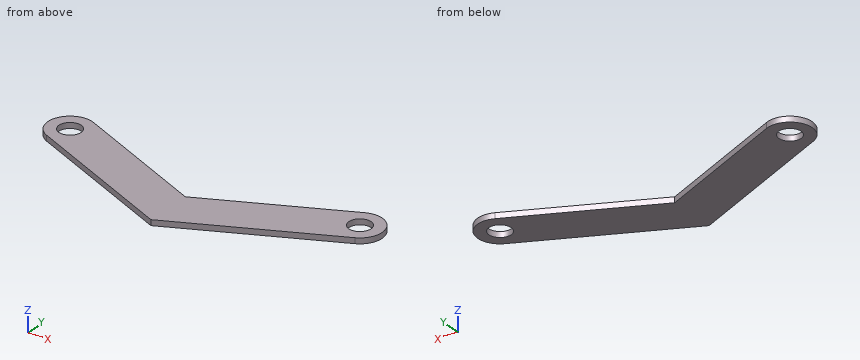
from build123d import *

# Parameters (mm, degrees)
SKETCH1_R           = 5
BOSS_EXTRUDE1_DEPTH = 2.5


with BuildPart() as part:
    # Sketch1 → Boss-Extrude1 (new body)
    with BuildSketch(Plane.XY):
        with BuildLine():
            Line((0, 21.995608), (61.387985551, 50.094742382))
            ThreePointArc((61.387985551, 50.094742382), (74.642724329, 45.164032502), (69.712014449, 31.909293724))
            Line((69.712014449, 31.909293724), (0, 0))
            Line((0, 0), (-69.712014449, 31.909293724))
            ThreePointArc((-69.712014449, 31.909293724), (-74.642724329, 45.164032502), (-61.387985551, 50.094742382))
            Line((-61.387985551, 50.094742382), (0, 21.995608))
        make_face()
        with Locations((-65.55, 41.002018053)):
            Circle(SKETCH1_R, mode=Mode.SUBTRACT)
        with Locations((65.55, 41.002018053)):
            Circle(SKETCH1_R, mode=Mode.SUBTRACT)
    extrude(amount=BOSS_EXTRUDE1_DEPTH)


solid = part.part
Geometry check sheet. Reference: the model listing, model coordinates, mm. Give positions to 0.01 mm unless a question says otherwise; leave off trailing zeros. Write each loop counter-clockwise with the first axis right and the second up, starting at its lowest first coordinate (ties: lowest second). Pieces come first, ordered by that corner, then holes.
1) Cross-section at B-B (z = 0.55). Record the boundary of the cut face in (x, y), plus the area to 3 significant figures.
Values follow:
outline: (-69.71, 31.91) - (0, 0) - (69.71, 31.91) arc R10 ccw to (61.39, 50.09) - (0, 22) - (-61.39, 50.09) arc R10 ccw to start; hole circle Ø10 at (-65.55, 41); hole circle Ø10 at (65.55, 41)
area: 3,040 mm2
2) Cross-section at D-D (x = -65.55). Record the boundary of the cut face in (y, z).
Values follow:
outline: (30, 0) - (36, 0) - (36, 2.5) - (30, 2.5) - close; (46, 0) - (51, 0) - (51, 2.5) - (46, 2.5) - close
3) Thickness scan on line 1 (X direction, y = 42, z = 0.85); line 2 (X direction, y = 47, z = 1.95); line 3 (Y direction, x = -65.55, z = 1.5). Record the ranges inside material, lowest first.
Values follow:
line 1: x = -75.5 to -70.45, -60.65 to -43.7, 43.7 to 60.65, 70.45 to 75.5
line 2: x = -73.55 to -54.63, 54.63 to 73.55
line 3: y = 30 to 36, 46 to 51
4) Cross-section at C-C (y = 44.5). Record the boundary of the cut face in (x, z).
Values follow:
outline: (-74.92, 0) - (-69.12, 0) - (-69.12, 2.5) - (-74.92, 2.5) - close; (-61.98, 0) - (-49.17, 0) - (-49.17, 2.5) - (-61.98, 2.5) - close; (49.17, 0) - (61.98, 0) - (61.98, 2.5) - (49.17, 2.5) - close; (69.12, 0) - (74.92, 0) - (74.92, 2.5) - (69.12, 2.5) - close
5) Go/stop test with flat-tipped pins: pin 1 Ø1.5 at (x, z) = (-38, 2) entering from +Y; pin 2 Ø10 at (x, y) = (49.5, 12) entering from +Z; pin 3 Ø16 at (x, y) = (65.55, 41) entering from -Z; pin 4 Ø1.5 at (y, z) = (39, 0.5) entering from -X. Record where each tip stops, or that it passes through.
Values follow:
pin 1: stops at y = 39.73
pin 2: passes through
pin 3: stops at z = 0
pin 4: stops at x = -75.47
6) Cross-section at A-A (x = 63). Record the boundary of the cut face in (y, z).
Values follow:
outline: (28.84, 0) - (36.7, 0) - (36.7, 2.5) - (28.84, 2.5) - close; (45.3, 0) - (50.67, 0) - (50.67, 2.5) - (45.3, 2.5) - close
